from build123d import *

# Parameters (mm, degrees)
SKETCH1_R        = 17.5
BASENUT_DEPTH    = 34.7
ENDCHAMFER2_SIZE = 1.156666667


with BuildPart() as part:
    # Sketch1 → BaseNut (new body)
    with BuildSketch(Plane.XY):
        Polygon((15.877132403, -27.5), (31.754264805, 0), (15.877132403, 27.5), (-15.877132403, 27.5), (-31.754264805, 0), (-15.877132403, -27.5), align=None)
        Circle(SKETCH1_R, mode=Mode.SUBTRACT)
    extrude(amount=-BASENUT_DEPTH)

    # Sketch2 → Chamfer1 (revolve, cut)
    with BuildSketch(Plane(origin=(15.04811501, 0, -16.706149795), x_dir=(0, 0, -1), z_dir=(0, 1, 0))):
        Polygon((15.537649274, 46.802379815), (17.993850205, 42.54811501), (17.993850205, 46.802379815), align=None)
    revolve(axis=Axis((0, 0, 7.016501752), (0, 0, -1)), mode=Mode.SUBTRACT)

    # Sketch6 → EndChamfer1 (revolve, cut)
    with BuildSketch(Plane(origin=(-9.197458863, 0, -10.252541137), x_dir=(0, 0, 1), z_dir=(0, 1, 0))):
        Polygon((-24.447458863, 26.697458863), (-24.447458863, 28.647458863), (-23.321625838, 26.697458863), align=None)
    revolve(axis=Axis((0, 0, 13.104863586), (0, 0, -1)), mode=Mode.SUBTRACT)

    # Sketch5 → Chamfer2 (revolve, cut)
    with BuildSketch(Plane(origin=(-14.793032735, 0, -16.96123207), x_dir=(0, 0, 1), z_dir=(0, 1, 0)), mode=Mode.PRIVATE) as chamfer2_sk:
        Polygon((16.96123207, 40.343032735), (16.96123207, 46.547297541), (13.379198115, 46.547297541), align=None)
    revolve(chamfer2_sk.sketch.rotate(Axis((0, 0, -39.536013381), (0, 0, 1)), 180), axis=Axis((0, 0, -39.536013381), (0, 0, 1)), mode=Mode.SUBTRACT)

    # EndChamfer2
    endchamfer2_edges = [part.edges().sort_by_distance(p)[0] for p in [
        (-17.5, 0, 0),
    ]]
    chamfer(endchamfer2_edges, length=ENDCHAMFER2_SIZE)


solid = part.part
Design review of the part built by this model. Coordinates are the model's own, in mm. Round coordinates to 2 decimals unless told otherwise and drop trailing zeros. Write each loop counter-clockwise with the first axis right and the second up, starting at its lowest first coordinate (ties: lowest second). Pieces come first, ordered by that corner, then holes. Notation, with made-up numbers: (71, 73) - (111, 73) arc R22 cw to (111, 92) - close; hole circle Ø2 at (46, -26.5). An arc over 180 degrees is marked (long way). Return JSON: item names as keys, results as strings. Group by question number.
Item 1: The part is to be moulded in two halves that separate along Y. For faces 1 (the face through (-23.9, -13.6, -17.7)), 2 (the face through (2, -19, 0)), 3 (the face through (-13.887, -10.648, -17.138)), 4 (the face through (23.9, 13.6, -17.7)), say which applies: pulls with the +Y half, pulls with the -Y half, needs draft (parallel to the pull), parting line crosses it, or undercut.
Item 2: We need section A-A on z = -20. Write out the cut boundary in (x, y), and give its area (3 significant figures).
Item 3: For probe 1 along Y at (x, z) = (0, -16.5); probe 2 along X at (y, z) = (0, -19); probe 3 along Y at (x, z) = (-12, -12), list the stretches that pass through material, from the lowest coordinate up. Write a range as [from, to].
Item 4: Insertion check: P1, Ø8, axis at x = 22.5, z = -24.5, coming from the -Y side; P2, Ø8, axis at y = 5.5, z = -9, coming from the +X side; P3, Ø1, axis at y = 14, z = -21, coming from the -X side. Each pin has a flat end and moves straight along its axis. Give the tip position at first contact, or say it passes through.
Model answer:
{
 "1": {"face 1": "pulls with the -Y half", "face 2": "needs draft", "face 3": "undercut", "face 4": "pulls with the +Y half"},
 "2": {"outline": "(-31.75, 0) - (-15.88, -27.5) - (15.88, -27.5) - (31.75, 0) - (15.88, 27.5) - (-15.88, 27.5) - close; hole circle Ø35 at (0, 0)", "area": "1,660 mm²"},
 "3": {"probe 1": "y = [-27.5, -17.5], [17.5, 27.5]", "probe 2": "x = [-31.75, -17.5], [17.5, 31.75]", "probe 3": "y = [-27.5, -12.74], [12.74, 27.5]"},
 "4": {"P1": "stops at y = -22.96", "P2": "stops at x = 30.89", "P3": "stops at x = -23.96"}
}
